Here's the drawing with two shaded views (mm, measured from the low corner). I have some questions. A direction names the side the tool comes from. Give positions to 0.01 mm unless a question says otherwise; leave off trailing zeros. Loops run counter-clockwise (first coordinate to the right, second up) from the corner with the lowest first, then second, coordinate; pieces in that order, holes last. Notation, with made-up numbers: M -38,88 L -12,88 A12 cw -12,101 Z; hole C -25,70.25 d9. An arc over 180 degrees is marked long. Put each result on its own line as item: value. Start each with the question number.
1) If we mould it in two halves opening along X, with no side actions, what happens to the marked faces 5, 6, 7 and 8? For each: +X half, -X half, draft (parallel to the pull), parting line (faces both ways), or undercut.
2) Please list where these lines run through material, in increasing order: line 1 along Y through (x, z) = (90, 30); line 2 along Y through (x, z) = (90, 2); line 3 along Z through (x, y) = (35, 9). Write a range as from..to.
3) Imagine slicing it at A-A (z = 61). Write out the boundary of the cut face in (x, y).
4) Imagine slicing it at C-C (z = 30). Write out the boundary of the cut face in (x, y), then the cut area to 3 significant figures.
5) For the marked faces 1, 2, 3 and 4, which set-ups out of +Z, -Z, +X, -X, +Y, -Y let a thin tool reach every point of the face, with its end or its side?
6) For P1, Ø6, axis at y = 75.5, z = 16.5, coming from the +X side; P2, Ø1.5, axis at y = 108, z = 33.5, coming from the +X side; P3, Ø4, axis at x = 18, z = 58.5, coming from the -Y side; P4, Ø3, axis at x = 46.5, y = 80, coming from the +Z side, each with a flat end and sliding along its axis, tell me the tip position at first contact or that it passes through.
7) Imagine slicing it at B-B (x = 90). Write out the boundary of the cut face in (y, z), then the cut area to 3 significant figures.
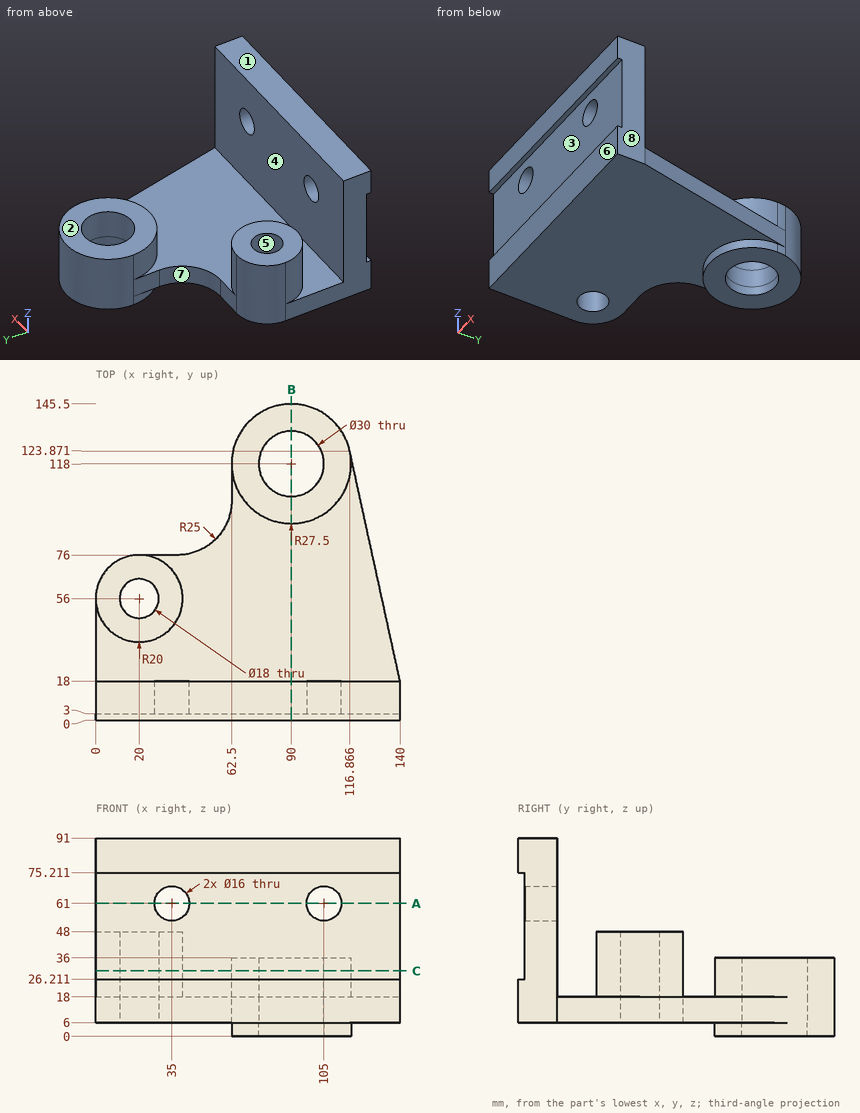
Recorded:
1. face 5: undercut
1. face 6: draft
1. face 7: -X half
1. face 8: +X half
2. line 1: 3..18, 90.5..103, 133..145.5
2. line 2: 90.5..103, 133..145.5
2. line 3: 6..53, 69..91
3. outline: M 0,3 L 27,3 L 27,18 L 0,18 Z; M 43,3 L 97,3 L 97,18 L 43,18 Z; M 113,3 L 140,3 L 140,18 L 113,18 Z
4. outline: M 0,3 L 140,3 L 140,18 L 0,18 Z; C 20,56 d40; C 90,118 d55; hole C 20,56 d18; hole C 90,118 d30
4. area: 4,770 mm²
5. face 1: +Z, +X, -X, +Y, -Y
5. face 2: +Z, +X, -X, +Y
5. face 3: +X, -X, -Y
5. face 4: +Z, +X, -X
6. P1: x = 128.09
6. P2: x = 115.9
6. P3: y = 3
6. P4: through
7. outline: M 0,6 L 90.5,6 L 90.5,0 L 103,0 L 103,36 L 90.5,36 L 90.5,18 L 18,18 L 18,91 L 0,91 L 0,75.21 L 3,75.21 L 3,26.21 L 0,26.21 Z; M 133,0 L 145.5,0 L 145.5,36 L 133,36 Z
7. area: 3,150 mm²
